Check sheet for the modelled part. Datum: model origin and axes. Units: mm. Round coordinates to 2 decimals unless told otherwise and drop trailing zeros. Loops run counter-clockwise (first coordinate to the right, second up) from the corner with the lowest first, then second, coordinate; pieces in that order, holes last. Notation, with made-up numbers: (69.25, 3) -> (93.25, 3) arc R26 cw to (93.25, 26) -> close; hole circle Ø1 at (-29.5, 24). An arc over 180 degrees is marked (long way). Use one line per item in the form item = value. Start each with the question number.
(1) Sectioned sample at D-D (y = 11). Record the cut outline in (x, z), and give its area (3 significant figures).
(2) Material ranges on probe 1 along Y at (x, z) = (20, -1); probe 2 along Y at (x, z) = (138, -0.5); probe 3 along X at (y, z) = (10, 0), recorded low to high. Write a range as [from, to].
(3) Sectioned sample at B-B (x = 20). Record the cut outline in (y, z), and give its area (3 significant figures).
(4) Sectioned sample at C-C (z = -2.75). Record the cut outline in (x, y), and give its area (3 significant figures).
(5) Sectioned sample at A-A (y = 55). Record the cut outline in (x, z).
(6) Go/stop test with flat-tipped pins: pin 1 (9.5 mm diameter, centred on x = 90, y = 55, fed in from -Z); pin 2 (3 mm diameter, centred on x = 166, z = 3, fed in from -Y); pin 3 (6 mm diameter, centred on y = 11, z = -1.5, fed in from +X). Record where each tip stops, or that it passes through.
from build123d import *

# Parameters (mm, degrees)
BOSS_EXTRUDE1_DEPTH        = 5
F_12_0_12_DIAMETER_HOLE1_D = 12


with BuildPart() as part:
    # Sketch1 → Boss-Extrude1 (new, symmetric)
    with BuildSketch(Plane.XY):
        Polygon((0, 0), (0, 90), (210, 90), (210, 20), (100, 20), (100, 0), align=None)
    extrude(amount=BOSS_EXTRUDE1_DEPTH, both=True)

    # Ø12.0 (12) Diameter Hole1 (through all)
    with Locations(Plane.XY.offset(5)):
        with Locations((20, 55), (90, 55)):
            Hole(F_12_0_12_DIAMETER_HOLE1_D / 2)


solid = part.part
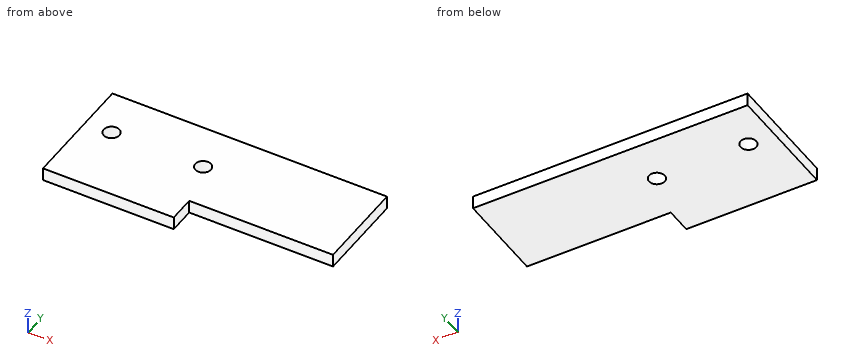
Checks:
q1.outline = (0, -5) -> (100, -5) -> (100, 5) -> (0, 5) -> close
q1.area = 1,000 mm2
q2.probe_1 = [0, 49], [61, 90]
q2.probe_2 = [20, 90]
q2.probe_3 = [0, 100]
q3.outline = (0, -5) -> (49, -5) -> (49, 5) -> (0, 5) -> close; (61, -5) -> (90, -5) -> (90, 5) -> (61, 5) -> close
q3.area = 780 mm2
q4.outline = (0, 0) -> (100, 0) -> (100, 20) -> (210, 20) -> (210, 90) -> (0, 90) -> close; hole circle Ø12 at (20, 55); hole circle Ø12 at (90, 55)
q4.area = 16,500 mm2
q5.outline = (0, -5) -> (14, -5) -> (14, 5) -> (0, 5) -> close; (26, -5) -> (84, -5) -> (84, 5) -> (26, 5) -> close; (96, -5) -> (210, -5) -> (210, 5) -> (96, 5) -> close
q6.pin_1 = through
q6.pin_2 = 20
q6.pin_3 = 100
